Here's the drawing with two shaded views (mm, measured from the low corner). I have some questions. A direction names the side the tool comes from. Give positions to 0.01 mm unless a question says otherwise; leave off trailing zeros. Loops run counter-clockwise (first coordinate to the right, second up) from the corner with the lowest first, then second, coordinate; pieces in that order, holes last. Notation, with made-up numbers: (85, 56) -> (123, 56) arc R22 cw to (123, 74) -> close; hole circle Ø8 at (-3.75, 49). An arc over 180 degrees is marked (long way). Answer in a Markdown table with one row per item. Add a question column.
Item 1: Which directions (+Z, -Z, +X, -X, +Y, -Y) give clear straight access to the entire face, cutting with the end or side of a thin tool? Please do the marked faces 1 and 2.
Item 2: If we section it at A-A (x = 12.5): Write out the boundary of the cut face in (y, z), then the cut area to 3 significant figures.
Item 3: For P1, Ø6, axis at x = 5.5, y = 24.5, coming from the -Z side; P2, Ø1, axis at x = 13, y = 7.5, coming from the -Z side; P3, Ø12, axis at y = 26.5, z = 19.5, coming from the -X side, each with a flat end and sliding along its axis, tell me the tip position at first contact or that it passes through.
Item 4: If I drill on line 1 (Y direction, x = 2, z = 15.75); line 2 (Z direction, x = 12.25, y = 18); line 3 (Z direction, x = 12.25, y = 4) (3 decimals), over which ranges is the centre line in solid material (lowest first)?
Item 5: If we section it at D-D (y = 32): Write out the boundary of the cut face in (x, z), then the cut area to 3 significant figures.
Item 6: If we section it at B-B (z = 12.5): Write out the boundary of the cut face in (x, y).
Item 7: If we section it at C-C (y = 19.5): Write out the boundary of the cut face in (x, z), then the cut area to 3 significant figures.
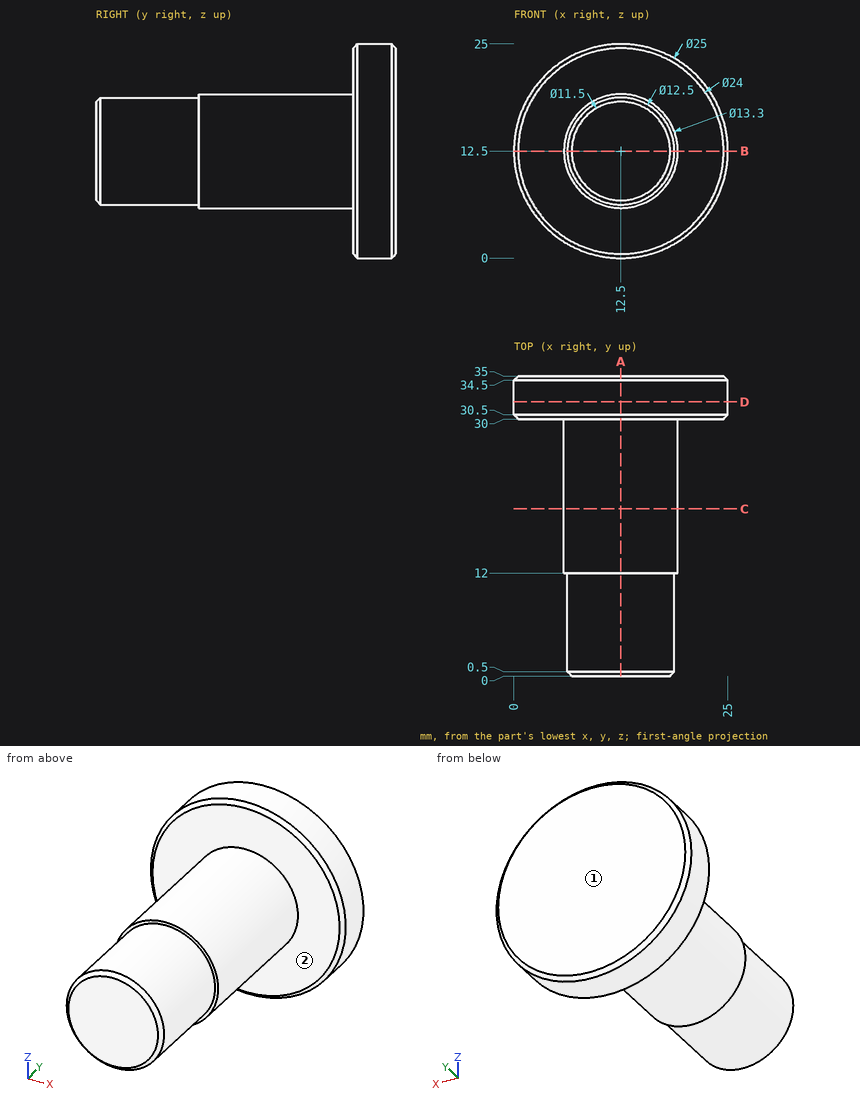
Recorded:
| question | item | result |
|---|---|---|
| 1 | face 1 | +Z, -Z, +X, -X, +Y |
| 1 | face 2 | -Y |
| 2 | outline | (0, 6.75) -> (0.5, 6.25) -> (12, 6.25) -> (12, 5.85) -> (30, 5.85) -> (30, 0.5) -> (30.5, 0) -> (34.5, 0) -> (35, 0.5) -> (35, 24.5) -> (34.5, 25) -> (30.5, 25) -> (30, 24.5) -> (30, 19.15) -> (12, 19.15) -> (12, 18.75) -> (0.5, 18.75) -> (0, 18.25) -> close |
| 2 | area | 514 mm^2 |
| 3 | P1 | stops at z = 7.19 |
| 3 | P2 | stops at z = 6.25 |
| 3 | P3 | stops at x = 0.26 |
| 4 | line 1 | y = 30 to 35 |
| 4 | line 2 | z = 5.85 to 19.15 |
| 4 | line 3 | z = 6.255 to 18.745 |
| 5 | outline | circle Ø25 at (12.5, 12.5) |
| 5 | area | 491 mm^2 |
| 6 | outline | (0, 30.5) -> (0.5, 30) -> (5.85, 30) -> (5.85, 12) -> (6.25, 12) -> (6.25, 0.5) -> (6.75, 0) -> (18.25, 0) -> (18.75, 0.5) -> (18.75, 12) -> (19.15, 12) -> (19.15, 30) -> (24.5, 30) -> (25, 30.5) -> (25, 34.5) -> (24.5, 35) -> (0.5, 35) -> (0, 34.5) -> close |
| 7 | outline | circle Ø13.3 at (12.5, 12.5) |
| 7 | area | 139 mm^2 |
